Could you check a few things on this model? Use its own coordinates, in mm. A direction names the side the tool comes from. Give positions to 0.01 mm unless a question says otherwise; leave off trailing zeros. Loops run counter-clockwise (first coordinate to the right, second up) from the corner with the lowest first, then second, coordinate; pieces in that order, holes last. Notation, with made-up numbers: (86, -6) -> (96, -6) arc R19 ccw to (96, 2) -> close; hole circle Ø7 at (25, -14.75). An arc over 180 degrees is marked (long way). Write item = value, one per line. Start each with the question number.
1) I want a section at A-A (x = 0). List the corners of the cut face in (y, z) for me, and give its area (3 significant figures).
2) I want a section at C-C (z = 15). List the corners of the cut face in (x, y) for me.
3) I need wall thicknesses on probe 1 along X at (y, z) = (0, 15); probe 2 along Y at (x, z) = (0, 22.25); probe 3 along Y at (x, z) = (0, 19.75). Which ranges of each line are inside material? Lowest first, please. Write a range as from..to.
4) On a 3-axis mill with a long thin cutter (end or side, diameter ignored), from which of +Z, -Z, +X, -X, +Y, -Y can I reach the whole of each face in a straight line? I mean faces 3 (the face through (-0.084, -57.596, 31.677)), 4 (the face through (18, -47, 20)), 5 (the face through (-18, -47, 20)). Say none if no direction works.
5) I'm going to push flat-ended pins straight in: pin 1 Ø10 at (x, z) = (14, 22) entering from +Y; pin 2 Ø2 at (x, y) = (2, -24) entering from +Z; pin 3 Ø4 at (x, z) = (-0.5, 26.5) entering from +Y. Where does each tip first touch, or does it pass through?
6) If we mould it in two halves opening along Y, with no side actions, what happens to faces 1 (the face through (0.42, -119.643, 18.252)), 2 (the face through (0, -37, 0))? For each: +Y half, -Y half, draft (parallel to the pull), parting line (faces both ways), or undercut.
7) I want a section at D-D (x = -24). List the corners of the cut face in (y, z) for me.
8) I want a section at B-B (y = -105). List the corners of the cut face in (x, z) for me, and give its area (3 significant figures).
from build123d import *

# Parameters (mm, degrees)
UPPER_EYE_SKETCH_R      = 30
UPPER_EYE_BOSS_DEPTH    = 30
UPPER_EYE_BORE_SKETCH_R = 15
UPPER_EYE_BORE_DEPTH    = 52.961524227
ARM_PROFILE_SKETCH_W    = 20
ARM_PROFILE_SKETCH_H    = 80
ARM_DEPTH               = 30
ARM_START               = 60
ARM_TRIM_CUT_DEPTH      = 60
LOWER_EYE_SKETCH_R      = 30
LOWER_EYE_BOSS_DEPTH    = 30
ARM_RIB_12MM_REACH      = 147.43
ARM_RIB_SKETCH_WALL_W   = 351.093498284
ARM_RIB_SKETCH_WALL_H   = 12
LOWER_EYE_BORE_SKETCH_R = 15
LOWER_EYE_BORE_DEPTH    = 155.434452115


with BuildPart() as part:
    # Upper Eye Sketch → Upper Eye Boss (new body)
    with BuildSketch(Plane.XY):
        Circle(UPPER_EYE_SKETCH_R)
    extrude(amount=UPPER_EYE_BOSS_DEPTH)

    # Upper Eye Bore Sketch → Upper Eye Bore (cut, through all)
    with BuildSketch(Plane.XY.offset(30)):
        Circle(UPPER_EYE_BORE_SKETCH_R)
    extrude(amount=-UPPER_EYE_BORE_DEPTH, mode=Mode.SUBTRACT)

    # Arm Profile Sketch → Arm (add, symmetric)
    with BuildSketch(Plane(origin=(0, 0, 0), x_dir=(0, 0, -1), z_dir=(1, 0, 0))):
        with Locations((-10, -40)):
            Rectangle(ARM_PROFILE_SKETCH_W, ARM_PROFILE_SKETCH_H)
    extrude(amount=ARM_DEPTH, both=True)

    # Arm Trim Sketch → Arm Trim Cut (cut)
    with BuildSketch(Plane.XY.offset(ARM_START)):
        with BuildLine():
            Line((15, 0), (-15, 0))
            ThreePointArc((-15, 0), (0, -15), (15, 0))
        make_face()
    extrude(amount=-ARM_TRIM_CUT_DEPTH, mode=Mode.SUBTRACT)

    # Lower Eye Sketch → Lower Eye Boss (add, symmetric)
    with BuildSketch(Plane(origin=(0, 0, 0), x_dir=(0, 0, -1), z_dir=(1, 0, 0))):
        with Locations((-15, -105)):
            Circle(LOWER_EYE_SKETCH_R)
    extrude(amount=LOWER_EYE_BOSS_DEPTH, both=True)

    # Arm Rib Sketch wall → Arm Rib 12mm (add, up to next)
    with BuildSketch(Plane(origin=(0, -58.299786749, 31.847196974), x_dir=(0, -0.971955050189, 0.235166707705), z_dir=(0, -0.235166707705, -0.971955050189)), mode=Mode.PRIVATE) as arm_rib_12mm_sk1:
        Rectangle(ARM_RIB_SKETCH_WALL_W, ARM_RIB_SKETCH_WALL_H)
    arm_rib_12mm_tool1 = extrude(arm_rib_12mm_sk1.sketch, amount=ARM_RIB_12MM_REACH, mode=Mode.PRIVATE) - part.part
    add(arm_rib_12mm_tool1.solids().sort_by_distance((0, -58.299786749, 31.847196974))[0])

    # Lower Eye Bore Sketch → Lower Eye Bore (cut, through all)
    with BuildSketch(Plane(origin=(30, 0, 0), x_dir=(0, 0, -1), z_dir=(1, 0, 0))):
        with Locations((-15, -105)):
            Circle(LOWER_EYE_BORE_SKETCH_R)
    extrude(amount=-LOWER_EYE_BORE_DEPTH, mode=Mode.SUBTRACT)


solid = part.part
Answer list:
q1.outline = (-86.6, 38.69) arc R30 ccw (long way) to (-79.02, 0) -> (-15, 0) -> (-15, 30) -> (-30, 30) -> (-30, 25) -> close; (15, 0) -> (30, 0) -> (30, 30) -> (15, 30) -> close; hole circle Ø30 at (-105, 15)
q1.area = 4,480 mm^2
q2.outline = (-30, -135) -> (30, -135) -> (30, -120) -> (-30, -120) -> close; (-30, -90) -> (30, -90) -> (30, 0) arc R30 ccw to (-30, 0) -> close; hole circle Ø30 at (0, 0)
q3.probe_1 = -30..-15, 15..30
q3.probe_2 = -134.11..-118.13, -91.87..-15, 15..30
q3.probe_3 = -134.62..-119.23, -90.77..-15, 15..30
q4.face_3 = +Z, +X, -X
q4.face_4 = +Z, +X
q4.face_5 = +Z, -X
q5.pin_1 = 28.62
q5.pin_2 = 30
q5.pin_3 = 30
q6.face_1 = undercut
q6.face_2 = draft
q7.outline = (-79.02, 0) -> (18, 0) -> (18, 30) -> (-18, 30) -> (-18, 20) -> (-75.42, 20) arc R30 ccw (long way) to start; hole circle Ø30 at (-105, 15)
q8.outline = (-30, -15) -> (30, -15) -> (30, 0) -> (-30, 0) -> close; (-30, 30) -> (30, 30) -> (30, 45) -> (-30, 45) -> close
q8.area = 1,800 mm^2
